Geometry: final body of the model. Coordinates: model frame, mm. Face numbers are marked on the shaded views. A direction names the side the tool comes from. Give positions to 0.01 mm unless a question says otherwise; leave off trailing zeros. Write each loop counter-clockwise with the first axis right and the second up, starting at its lowest first coordinate (ties: lowest second). Pieces come first, ordered by that corner, then holes. Notation, with made-up numbers: M 10,-12.75 L 45,-12.75 A14 cw 45,5.25 Z; hole C -34.5,-9.75 d1. An arc over 180 degrees is marked long. Use a Markdown table: item, result. Add a question column.
1) Section A-A on z = 40. Return the cut outline in (x, y), then the cut area to 3 significant figures.
2) Set-up query: the marked faces 1, 2, 3, 4 and 5. Return all of +Z, -Z, +X, -X, +Y, -Y with unobstructed straight access to the full face (end or side cutting, diameter ignored); none if empty.
3) Line query: line 1 (Y direction, x = 0, z = 2); line 2 (Z direction, x = -19.5, y = 44); line 3 (X direction, y = 20, z = 34.5). Output: solid intervals per line, ascending.
4) Pin query (flat end, axial travel): pin 1 (5 mm diameter, centred on x = 35, y = 24, fed in from -Z); pin 2 (12 mm diameter, centred on x = -19, y = 24.5, fed in from +Z); pin 3 (6 mm diameter, centred on x = 35, z = 13.5, fed in from -Y); pin 4 (2 mm diameter, centred on y = 24, z = 12.5, fed in from -X). Return the tip coordinate at first contact, or that it passes through.
5) Section B-B on y = 45. Return the cut outline in (x, z).
6) Draft query along Y for the marked faces 6, 7 and 8. Return one class per face: +Y half, -Y half, draft (parallel to the pull), parting line (faces both ways), or undercut.
7) Section D-D on x = -3.5. Return the cut outline in (y, z), then the cut area to 3 significant figures.
```python
from build123d import *

# Parameters (mm, degrees)
LUG_PLATE_DEPTH          = 10
FLANGE_BASE_DEPTH        = 10
ANGLED_FLANGE_ARMS_DEPTH = 22
EYE_BOSS_A_SKETCH_R      = 18.000000011
EYE_BOSS_A_DEPTH         = 10
EYE_BOSS_B_SKETCH_R      = 18
EYE_BOSS_B_DEPTH         = 10
EYE_HOLE_A_22_SKETCH_R   = 11
EYE_HOLE_A_22_DEPTH      = 10
EYE_HOLE_B_22_SKETCH_R   = 11
EYE_HOLE_B_22_DEPTH      = 10
LUG_BORE_25_SKETCH_R     = 12.5
LUG_BORE_25_DEPTH        = 10


with BuildPart() as part:
    # Lug Plate Sketch → Lug Plate (new body)
    with BuildSketch(Plane.XY):
        with BuildLine():
            Line((-19.074339015, 51.01411599), (-32.420050634, 8.686926386))
            Line((-32.420050634, 8.686926386), (0, 0))
            Line((0, 0), (32.420050634, 8.686926386))
            Line((32.420050634, 8.686926386), (19.074339015, 51.01411599))
            ThreePointArc((19.074339015, 51.01411599), (0, 65), (-19.074339015, 51.01411599))
        make_face()
    extrude(amount=LUG_PLATE_DEPTH)

    # Flange Base Sketch → Flange Base (add)
    with BuildSketch(Plane.XY.offset(10)):
        Polygon((-54.079171789, 14.541040303), (-32.414511502, 8.704494269), (-29.410127859, 18.233181813), (-51.490581609, 24.149621564), align=None)
        Polygon((-32.414511502, 8.704494269), (-19.318516526, 5.176380902), (-16.730326075, 14.835639165), (-29.410127859, 18.233181813), align=None)
        Polygon((16.730326075, 14.835639165), (19.318516526, 5.176380902), (32.420050634, 8.686926386), (29.410127859, 18.233181813), align=None)
        Polygon((29.410127859, 18.233181813), (32.420050634, 8.686926386), (54.091846272, 14.493866526), (51.503655821, 24.153124789), align=None)
    extrude(amount=-FLANGE_BASE_DEPTH)

    # Angled Flange Arms Sketch → Angled Flange Arms (add)
    with BuildSketch(Plane.XY.offset(10)):
        Polygon((-51.490581609, 24.149621564), (-16.729926347, 14.784962163), (-19.318186451, 5.177606105), (-54.079171789, 14.541040303), align=None)
        Polygon((51.503655821, 24.153124789), (16.730326075, 14.835639165), (19.318516526, 5.176380902), (54.091846272, 14.493866526), align=None)
    extrude(amount=ANGLED_FLANGE_ARMS_DEPTH)

    # Eye Boss A Sketch → Eye Boss A (add)
    with BuildSketch(Plane(origin=(-0.006544851, -0.024297225, 0), x_dir=(0.965582925438563, -0.2600953942335516, 0), z_dir=(-0.2600953942335516, -0.9655829254385631, 0))):
        with Locations((-37.9999825, 32)):
            Circle(EYE_BOSS_A_SKETCH_R)
    extrude(amount=-EYE_BOSS_A_DEPTH)

    # Eye Boss B Sketch → Eye Boss B (add)
    with BuildSketch(Plane(origin=(0, 0, 0), x_dir=(0.9659258262890681, 0.25881904510252146, 0), z_dir=(0.25881904510252146, -0.9659258262890681, 0))):
        with Locations((38, 32)):
            Circle(EYE_BOSS_B_SKETCH_R)
    extrude(amount=-EYE_BOSS_B_DEPTH)

    # Eye Hole A _22 Sketch → Eye Hole A _22 (cut)
    with BuildSketch(Plane(origin=(-0.006544851, -0.024297225, 0), x_dir=(0.965582925438563, -0.2600953942335516, 0), z_dir=(-0.2600953942335516, -0.9655829254385631, 0))):
        with Locations((-37.9999825, 32)):
            Circle(EYE_HOLE_A_22_SKETCH_R)
    extrude(amount=-EYE_HOLE_A_22_DEPTH, mode=Mode.SUBTRACT)

    # Eye Hole B _22 Sketch → Eye Hole B _22 (cut)
    with BuildSketch(Plane(origin=(0, 0, 0), x_dir=(0.9659258262890681, 0.25881904510252146, 0), z_dir=(0.25881904510252146, -0.9659258262890681, 0))):
        with Locations((38, 32)):
            Circle(EYE_HOLE_B_22_SKETCH_R)
    extrude(amount=-EYE_HOLE_B_22_DEPTH, mode=Mode.SUBTRACT)

    # Lug Bore _25 Sketch → Lug Bore _25 (cut)
    with BuildSketch(Plane.XY.offset(10)):
        with Locations((0, 45)):
            Circle(LUG_BORE_25_SKETCH_R)
    extrude(amount=-LUG_BORE_25_DEPTH, mode=Mode.SUBTRACT)


solid = part.part
```
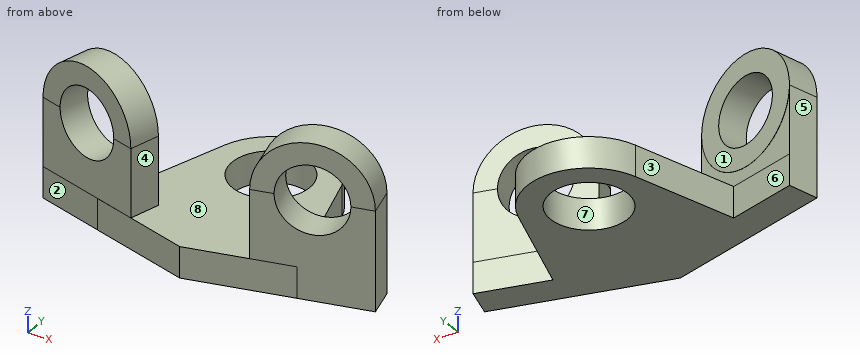
Found:
| question | item | result |
|---|---|---|
| 1 | outline | M -52.27,14.05 L -43.99,11.82 L -41.39,21.48 L -49.67,23.71 Z; M -29.41,7.9 L -21.13,5.67 L -18.53,15.32 L -26.81,17.55 Z; M 18.54,15.32 L 21.13,5.66 L 29.41,7.88 L 26.82,17.54 Z; M 41.41,21.45 L 44,11.79 L 52.28,14.01 L 49.69,23.67 Z |
| 1 | area | 343 mm² |
| 2 | face 1 | +Z, +Y |
| 2 | face 2 | +Z, -Z, -X, -Y |
| 2 | face 3 | +Z, -Z, +Y |
| 2 | face 4 | +Z, -Y |
| 2 | face 5 | +Z, -Z, -X, +Y |
| 3 | line 1 | 0 to 32.5, 57.5 to 65 |
| 3 | line 2 | 0 to 10 |
| 3 | line 3 | -52.43 to -45.06, 45.07 to 52.44 |
| 4 | pin 1 | through |
| 4 | pin 2 | z = 10 |
| 4 | pin 3 | y = 8.57 |
| 4 | pin 4 | x = -51.8 |
| 5 | outline | M -20.97,0 L -12.5,0 L -12.5,10 L -20.97,10 Z; M 12.5,0 L 20.97,0 L 20.97,10 L 12.5,10 Z |
| 6 | face 6 | +Y half |
| 6 | face 7 | undercut |
| 6 | face 8 | draft |
| 7 | outline | M 0.94,0 L 33,0 L 33,10 L 0.94,10 Z; M 57,0 L 64.69,0 L 64.69,10 L 57,10 Z |
| 7 | area | 398 mm² |
